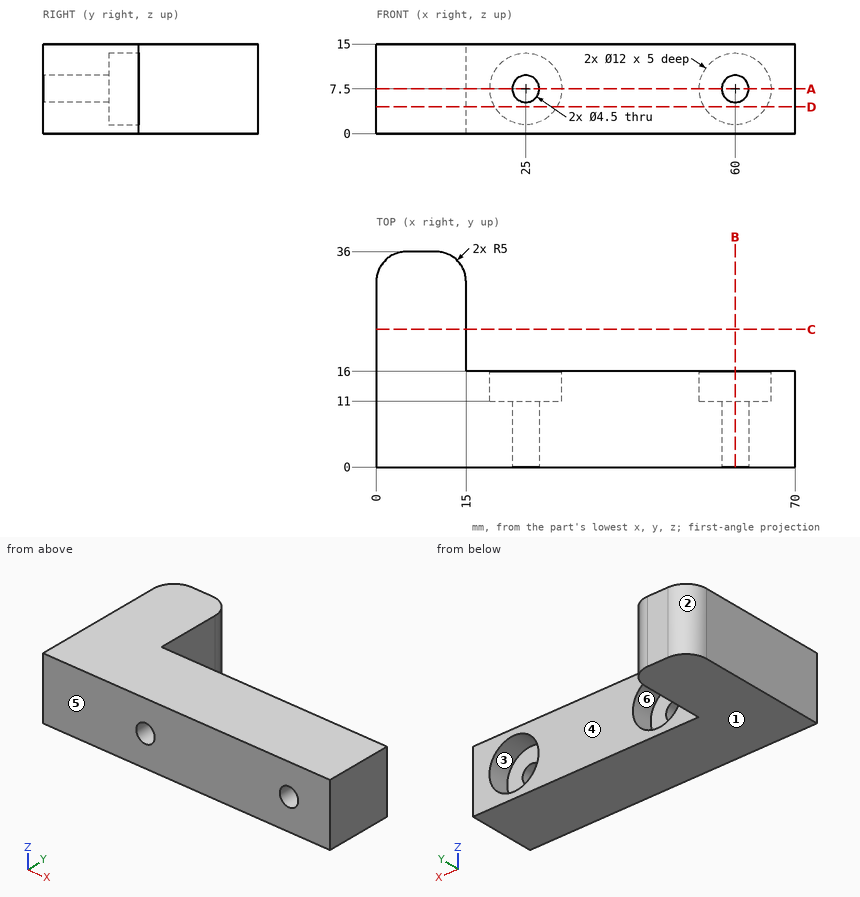
Can you work these out from the drawing? Everything is in mm from the part's minimum corner. A direction names the side the tool comes from. Coordinates: 2 decimals unless noted, no trailing zeros. Write each loop counter-clockwise with the first axis right and the second up, starting at its lowest first coordinate (ties: lowest second). Pieces come first, ordered by that corner, then holes. Notation, with made-up numbers: (-23, 69) -> (10, 69) arc R18 cw to (10, 102) -> close; hole circle Ø9 at (1, 48.5). An arc over 180 degrees is marked (long way). Write item = value, one per line.
(1) On a 3-axis mill with a long thin cutter (end or side, diameter ignored), from which of +Z, -Z, +X, -X, +Y, -Y can I reach the whole of each face in a straight line? I mean the marked faces 4, 5 and 6. Say none if no direction works.
Verdict:
face_4 = +Z, -Z, +X, +Y
face_5 = +Z, -Z, +X, -X, -Y
face_6 = +Y
(2) If I drill on probe 1 along Z at (x, y) = (25, 3); probe 2 along X at (y, z) = (12, 9.5); probe 3 along X at (y, z) = (21, 7.75), over which ranges is the centre line in solid material (lowest first)?
Verdict:
probe_1 = 0 to 5.25, 9.75 to 15
probe_2 = 0 to 19.34, 30.66 to 54.34, 65.66 to 70
probe_3 = 0 to 15
(3) For pin 1 (2 mm diameter, centred on x = 54.5, y = 17.5, fed in from -Z); pin 2 (4.5 mm diameter, centred on y = 24, z = 7.5, fed in from +X); pin 3 (3 mm diameter, centred on x = 52, z = 2.5, fed in from +Y); pin 4 (3.5 mm diameter, centred on x = 62, z = 8.5, fed in from +Y), each with a flat end and sliding along its axis, tell me the tip position at first contact or that it passes through.
Verdict:
pin_1 = through
pin_2 = 15
pin_3 = 16
pin_4 = 11
(4) Thinking about a two-plate mould opening in X: for the marked faces 1, 2 and 3, which applies, +X half, -X half, draft (parallel to the pull), parting line (faces both ways), or undercut?
Verdict:
face_1 = draft
face_2 = -X half
face_3 = undercut
(5) Imagine slicing it at C-C (y = 23). Please give me the cut outline in (x, z).
Verdict:
outline = (0, 0) -> (15, 0) -> (15, 15) -> (0, 15) -> close
(6) Imagine slicing it at D-D (z = 4.5). Please give me the cut outline in (x, y), and give its area (3 significant figures).
Verdict:
outline = (0, 0) -> (70, 0) -> (70, 16) -> (65.2, 16) -> (65.2, 11) -> (54.8, 11) -> (54.8, 16) -> (30.2, 16) -> (30.2, 11) -> (19.8, 11) -> (19.8, 16) -> (15, 16) -> (15, 31) arc R5 ccw to (10, 36) -> (5, 36) arc R5 ccw to (0, 31) -> close
area = 1,310 mm^2
(7) Imagine slicing it at A-A (z = 7.5). Please give me the cut outline in (x, y), and give its area (3 significant figures).
Verdict:
outline = (0, 0) -> (22.75, 0) -> (22.75, 11) -> (19, 11) -> (19, 16) -> (15, 16) -> (15, 31) arc R5 ccw to (10, 36) -> (5, 36) arc R5 ccw to (0, 31) -> close; (27.25, 0) -> (57.75, 0) -> (57.75, 11) -> (54, 11) -> (54, 16) -> (31, 16) -> (31, 11) -> (27.25, 11) -> close; (62.25, 0) -> (70, 0) -> (70, 16) -> (66, 16) -> (66, 11) -> (62.25, 11) -> close
area = 1,190 mm^2
(8) Imagine slicing it at B-B (x = 60). Please give me the cut outline in (y, z), and give its area (4 significant figures).
Verdict:
outline = (0, 0) -> (16, 0) -> (16, 1.5) -> (11, 1.5) -> (11, 5.25) -> (0, 5.25) -> close; (0, 9.75) -> (11, 9.75) -> (11, 13.5) -> (16, 13.5) -> (16, 15) -> (0, 15) -> close
area = 130.5 mm^2
